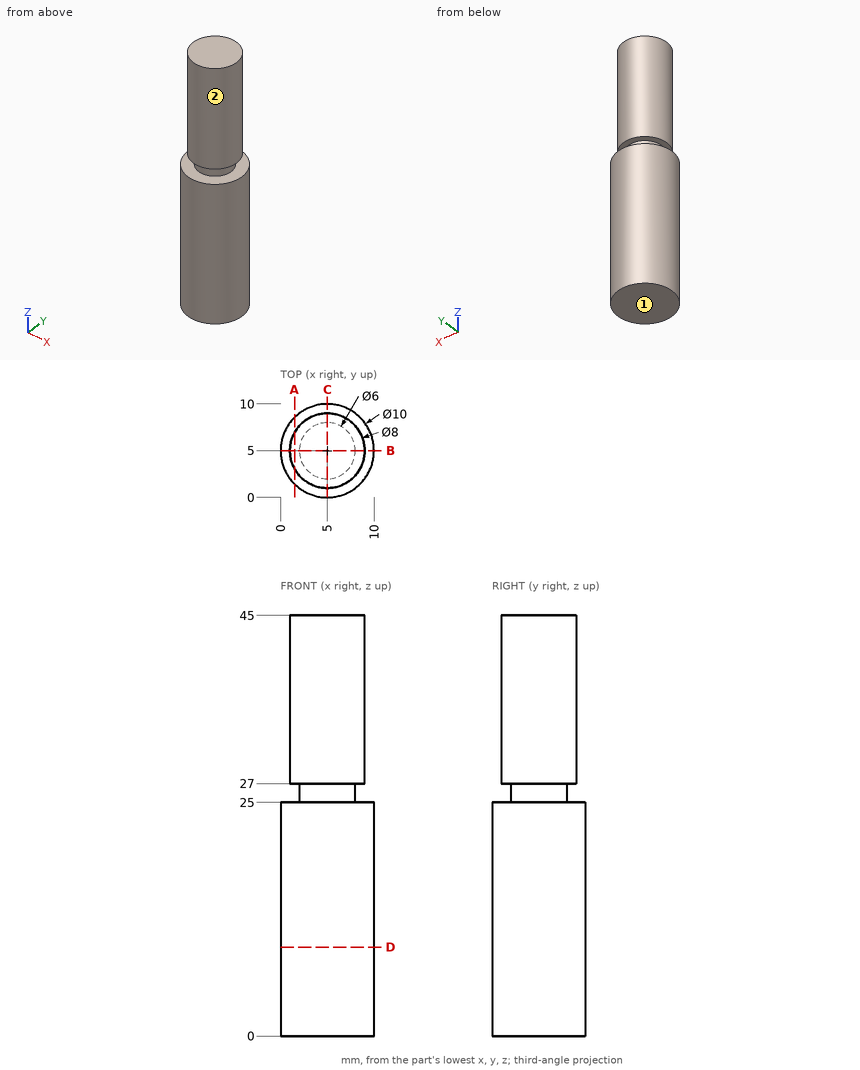
Design review of the part shown in the three views and the two pictorial views. Dimensions are in mm from the part's minimum x, y and z. A direction names the side the tool comes from. Round coordinates to 2 decimals unless told otherwise and drop trailing zeros. Loops run counter-clockwise (first coordinate to the right, second up) from the corner with the lowest first, then second, coordinate; pieces in that order, holes last. Notation, with made-up numbers: (-14.75, 54.25) - (25.25, 54.25) arc R25 ccw to (25.25, 92.25) - close; hole circle Ø9 at (84.5, -11). An arc over 180 degrees is marked (long way). One line per item, written item: value. Start each with the question number.
Item 1: For L1, parallel to Z at x = 8.25, y = 2.75; L2, parallel to Z at x = 0.75, y = 6.75; L3, parallel to X at y = 9, z = 19.5, list the stretches that pass through material, from the lowest coordinate up.
Item 2: Take a section at D-D (z = 9.5). Give the boundary of the cut face in (x, y).
Item 3: Take a section at A-A (x = 1.5). Give the boundary of the cut face in (y, z), plus the area to 3 significant figures.
Item 4: Clearance check with flat-ended pins moving along their axes: pin 1 Ø2 at (x, z) = (7.5, 25) entering from -Y; pin 2 Ø4 at (x, z) = (3, 24.5) entering from -Y; pin 3 Ø2 at (y, z) = (9, 19) entering from -X; pin 4 Ø1.5 at (x, z) = (8.5, 35.5) entering from +Y. State where each tip first meets the part, or that it passes through.
Item 5: Take a section at B-B (y = 5). Give the boundary of the cut face in (x, z).
Item 6: For the marked faces 1 and 2, list the 3-axis set-ups (+Z, -Z, +X, -X, +Y, -Y) from which the entire face can be reached by the end or side of a thin tool; tool diameter is ignored.
Answer below:
1. L1: z = 0 to 25, 27 to 45
1. L2: z = 0 to 25
1. L3: x = 2 to 8
2. outline: circle Ø10 at (5, 5)
3. outline: (1.43, 0) - (8.57, 0) - (8.57, 25) - (1.43, 25) - close; (3.06, 27) - (6.94, 27) - (6.94, 45) - (3.06, 45) - close
3. area: 248 mm2
4. pin 1: stops at y = 0.23
4. pin 2: stops at y = 0
4. pin 3: stops at x = 1
4. pin 4: stops at y = 7.9
5. outline: (0, 0) - (10, 0) - (10, 25) - (8, 25) - (8, 27) - (9, 27) - (9, 45) - (1, 45) - (1, 27) - (2, 27) - (2, 25) - (0, 25) - close
6. face 1: -Z, +X, -X, +Y, -Y
6. face 2: +Z
